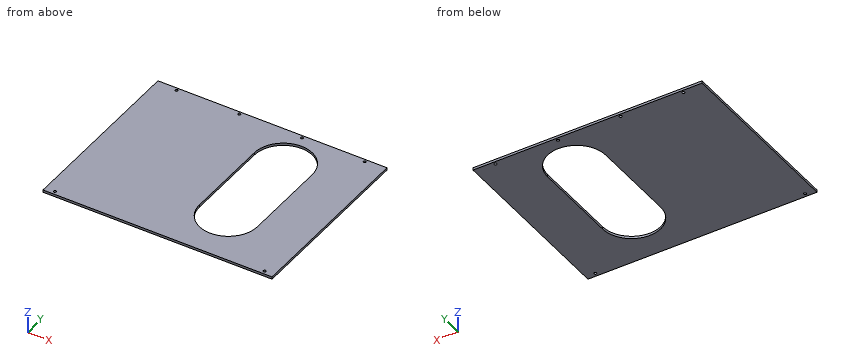
```python
from build123d import *

# Parameters (mm, degrees)
SKETCH1_W            = 475
SKETCH1_H            = 377
BOSS_EXTRUDE1_DEPTH  = 5
M5_CLEARANCE_HOLE1_D = 5.5
CUT_EXTRUDE1_DEPTH   = 10


with BuildPart() as part:
    # Sketch1 → Boss-Extrude1 (new body)
    with BuildSketch(Plane.XY):
        Rectangle(SKETCH1_W, SKETCH1_H)
    extrude(amount=BOSS_EXTRUDE1_DEPTH)

    # M5 Clearance Hole1 (through all)
    with Locations(Plane(origin=(0, 0, 0), x_dir=(-1, 0, 0), z_dir=(0, 0, -1))):
        with Locations((-195, 182.5), (-65, 182.5), (65, 182.5), (195, 182.5), (217.5, -181), (-217.5, -181)):
            Hole(M5_CLEARANCE_HOLE1_D / 2)

    # Sketch3 → Cut-Extrude1 (cut)
    with BuildSketch(Plane(origin=(0, 0, 0), x_dir=(-1, 0, 0), z_dir=(0, 0, -1))):
        with BuildLine():
            Line((-17.5, 101.5), (-17.5, -78.5))
            ThreePointArc((-17.5, -78.5), (-77.5, -138.5), (-137.5, -78.5))
            Line((-137.5, -78.5), (-137.5, 101.5))
            ThreePointArc((-137.5, 101.5), (-77.5, 161.5), (-17.5, 101.5))
        make_face()
    extrude(amount=-CUT_EXTRUDE1_DEPTH, mode=Mode.SUBTRACT)


solid = part.part
```
The model under review builds one solid part; all positions refer to its coordinate system, in mm. Round coordinates to 2 decimals unless told otherwise and drop trailing zeros. Order: outer loops, then holes, each group sorted by start corner. A loop starts at its lowest first (then second) coordinate and runs counter-clockwise, first axis right, second up. Notation, with made-up numbers: (33, -35) - (65, -35) arc R23 cw to (65, 1) - close; hole circle Ø6 at (-23, -30). An arc over 180 degrees is marked (long way). Answer in a Markdown table with one row per item.
(1) For line 1 (X direction, y = -181, z = 3.35); line 2 (X direction, y = 40, z = 2); line 3 (Y direction, x = 195, z = 1.9), list the stretches that pass through material, from the lowest coordinate up. Write a range as from..to.
Result set:
| item | result |
|---|---|
| line 1 | x = -237.5..-220.25, -214.75..214.75, 220.25..237.5 |
| line 2 | x = -237.5..17.5, 137.5..237.5 |
| line 3 | y = -188.5..179.75, 185.25..188.5 |
(2) Take a section at B-B on y = -70.5. Write out the cut boundary in (x, z).
Result set:
| item | result |
|---|---|
| outline | (-237.5, 0) - (17.5, 0) - (17.5, 5) - (-237.5, 5) - close; (137.5, 0) - (237.5, 0) - (237.5, 5) - (137.5, 5) - close |
(3) Take a section at C-C on x = 77.5. Write out the cut boundary in (y, z), plus the area to 3 significant figures.
Result set:
| item | result |
|---|---|
| outline | (-188.5, 0) - (-138.5, 0) - (-138.5, 5) - (-188.5, 5) - close; (161.5, 0) - (188.5, 0) - (188.5, 5) - (161.5, 5) - close |
| area | 385 mm2 |
(4) Take a section at A-A on z = 4.1. Write out the cut boundary in (x, y).
Result set:
| item | result |
|---|---|
| outline | (-237.5, -188.5) - (237.5, -188.5) - (237.5, 188.5) - (-237.5, 188.5) - close; hole circle Ø5.5 at (-217.5, -181); hole circle Ø5.5 at (-195, 182.5); hole circle Ø5.5 at (-65, 182.5); hole (17.5, -78.5) arc R60 ccw to (137.5, -78.5) - (137.5, 101.5) arc R60 ccw to (17.5, 101.5) - close; hole circle Ø5.5 at (65, 182.5); hole circle Ø5.5 at (195, 182.5); hole circle Ø5.5 at (217.5, -181) |
